```python
from build123d import *

# Parameters (mm, degrees)
SKETCH_1_W               = 1204
SKETCH_1_H               = 472
EXTRUDE_1_DEPTH          = 30
SHELL_1_T                = -2
SKETCH_2_W               = 1204
SKETCH_2_H               = 492
SKETCH_2_W_2             = 1164
SKETCH_2_H_2             = 450
EXTRUDE_2_DEPTH          = 2
CUT_EXTRUDE_1_DEPTH      = 1295
CUT_EXTRUDE_1_DEPTH_BACK = 72
SKETCH_3_R               = 4.5
SKETCH_4_R               = 4.5
CUT_EXTRUDE_2_DEPTH      = 45


with BuildPart() as part:
    # 草图1 → 凸台-拉伸1 (new body)
    with BuildSketch(Plane.XY):
        with Locations((602, 236)):
            Rectangle(SKETCH_1_W, SKETCH_1_H)
    extrude(amount=EXTRUDE_1_DEPTH)

    # 抽壳1
    shell_1_openings = [part.faces().sort_by_distance(p)[0] for p in [
        (602, 236, 30),
    ]]
    offset(amount=SHELL_1_T, openings=shell_1_openings, kind=Kind.INTERSECTION)

    # 草图2 → 凸台-拉伸2 (add)
    with BuildSketch(Plane.XY.offset(30)):
        with Locations((602, 246)):
            Rectangle(SKETCH_2_W, SKETCH_2_H)
        with Locations((602, 245)):
            Rectangle(SKETCH_2_W_2, SKETCH_2_H_2, mode=Mode.SUBTRACT)
    extrude(amount=-EXTRUDE_2_DEPTH)

    # 草图3 → 切除-拉伸1 (cut, two sides: drawn at the far end of the back side and taken through both)
    with BuildSketch(Plane(origin=(2, 0, 0), x_dir=(0, 0, -1), z_dir=(1, 0, 0)).offset(-CUT_EXTRUDE_1_DEPTH_BACK)):
        with Locations(Location((-16, 442, 0), (0, 0, 180))):
            Circle(SKETCH_3_R)
        with Locations(Location((-16, 30, 0), (0, 0, 180))):
            Circle(SKETCH_3_R)
    extrude(amount=CUT_EXTRUDE_1_DEPTH + CUT_EXTRUDE_1_DEPTH_BACK, mode=Mode.SUBTRACT)

    # 草图4 → 切除-拉伸2 (cut)
    with BuildSketch(Plane(origin=(0, 2, 0), x_dir=(1, 0, 0), z_dir=(0, 1, 0))):
        with Locations(Location((1174, -16, 0), (0, 0, 270))):
            Circle(SKETCH_4_R)
        with Locations(Location((30, -16, 0), (0, 0, 270))):
            Circle(SKETCH_4_R)
        with Locations(Location((1065, -16, 0), (0, 0, 270))):
            Circle(SKETCH_4_R)
        with Locations(Location((965, -16, 0), (0, 0, 270))):
            Circle(SKETCH_4_R)
        with Locations(Location((500, -16, 0), (0, 0, 270))):
            Circle(SKETCH_4_R)
    extrude(amount=-CUT_EXTRUDE_2_DEPTH, mode=Mode.SUBTRACT)


solid = part.part
```
Work out the finished part from the listing and answer in its coordinate system (mm). A direction names the side the tool comes from. Give positions to 0.01 mm unless a question says otherwise; leave off trailing zeros. Order: outer loops, then holes, each group sorted by start corner. A loop starts at its lowest first (then second) coordinate and runs counter-clockwise, first axis right, second up. Notation, with made-up numbers: M 73,-14.5 L 119,-14.5 A19 ccw 119,13.5 Z; hole C 89.25,-21.5 d2. An arc over 180 degrees is marked long. Return JSON: item names as keys, results as strings.
1) Section B-B, the plane x = 898.5 is taken. Write down the section's boundary in (y, z).
Resolved:
{"outline": "M 0,0 L 472,0 L 472,28 L 492,28 L 492,30 L 470,30 L 470,2 L 2,2 L 2,28 L 20,28 L 20,30 L 0,30 Z"}
2) Straight lines are drawn through the part: line 1 along X through (y, z) = (0.85, 16); line 2 along Y through (x, z) = (0.6, 16); line 3 along Y through (x, z) = (574, 8). For each, find the intervals that lie inside material, in ascending order. Write a range as [from, to].
Resolved:
{"line 1": "[0, 25.5], [34.5, 495.5], [504.5, 960.5], [969.5, 1060.5], [1069.5, 1169.5], [1178.5, 1204]", "line 2": "[0, 25.5], [34.5, 437.5], [446.5, 472]", "line 3": "[0, 2], [470, 472]"}
3) Section A-A, the plane y = 96 is taken. Write down the section's boundary in (x, z).
Resolved:
{"outline": "M 0,0 L 1204,0 L 1204,30 L 1184,30 L 1184,28 L 1202,28 L 1202,2 L 2,2 L 2,28 L 20,28 L 20,30 L 0,30 Z"}
4) For a pull along Z with two mould halves and no side action, classify faces 1 (the flat face through (421, 10, 30)), 2 (the flat face through (2, 233, 15)), 3 (the flat face through (594, 239, 0)), 4 (the flat face through (599, 12, 28)) as +Z half, -Z half, draft (parallel to the pull), parting line (faces both ways), or undercut.
Resolved:
{"face 1": "+Z half", "face 2": "undercut", "face 3": "-Z half", "face 4": "undercut"}
5) Each of these flat-tipped pins is pushed along its axis until it touches: pin 1 (6 mm diameter, centred on x = 436, y = 486, fed in from -Z); pin 2 (4 mm diameter, centred on x = 555.5, z = 12.5, fed in from +Y); pin 3 (12 mm diameter, centred on x = 651, y = 201, fed in from +Z); pin 4 (7 mm diameter, centred on y = 30, z = 16, fed in from +X). Where does it stop, or does it pass through?
Resolved:
{"pin 1": "z = 28", "pin 2": "y = 472", "pin 3": "z = 2", "pin 4": "through"}
6) A tool of negligible diameter and unlimited length cuts with its end or side. For faces 5 (the flat face through (594, 472, 14)), 6 (the flat face through (1202, 233, 15)), 7 (the flat face through (0, 243, 15)), from which of +Z, -Z, +X, -X, +Y, -Y can it reach the whole face along a straight path? Write none if from no direction.
Resolved:
{"face 5": "-Z, +X, -X, +Y", "face 6": "none", "face 7": "+Z, -Z, -X, +Y, -Y"}
7) Section C-C, the plane z = 16 is taken. Give the number of separate pieces and of enclosed holes in the cut face, plus the area to 3 significant figures.
Resolved:
{"separate pieces": "9", "enclosed holes": "0", "area": "6,530 mm^2"}
